The listing builds one solid part. Answer for the finished solid, in the listing's coordinates (mm). A direction names the side the tool comes from. Give positions to 0.01 mm unless a question says otherwise; leave off trailing zeros. Order: outer loops, then holes, each group sorted by start corner. A loop starts at its lowest first (then second) coordinate and runs counter-clockwise, first axis right, second up. Notation, with made-up numbers: (43, -11.75) -> (58, -11.75) arc R23 ccw to (58, 11.25) -> close; hole circle Ø6 at (-13.5, 48). An arc over 180 degrees is marked (long way). Write item = value, one per line. Start each with the question number.
```python
from build123d import *

# Parameters (mm, degrees)
SKETCH_1_W      = 130
SKETCH_1_H      = 130
SKETCH_1_R      = 5
EXTRUDE_1_DEPTH = 99
SKETCH_2_R      = 55
EXTRUDE_2_DEPTH = 5
SKETCH_3_R      = 11
EXTRUDE_3_DEPTH = 52
SKETCH_5_W      = 28.58431815
SKETCH_5_H      = 29.945476157
SKETCH_5_W_2    = 14.292159074
SKETCH_5_H_2    = 14.972738078
EXTRUDE_4_DEPTH = 86
SKETCH_6_R      = 40
EXTRUDE_5_DEPTH = 50


with BuildPart() as part:
    # 草图1 → 凸台-拉伸1 (new, symmetric)
    with BuildSketch(Plane.XY):
        Rectangle(SKETCH_1_W, SKETCH_1_H)
        with Locations((-51.265241636, 51.265241636)):
            Circle(SKETCH_1_R, mode=Mode.SUBTRACT)
        with Locations(Location((51.265241636, 51.265241636, 0), (0, 0, 180))):
            Circle(SKETCH_1_R, mode=Mode.SUBTRACT)
        with Locations(Location((-51.265241636, -51.265241636, 0), (0, 0, 180))):
            Circle(SKETCH_1_R, mode=Mode.SUBTRACT)
        with Locations((51.265241636, -51.265241636)):
            Circle(SKETCH_1_R, mode=Mode.SUBTRACT)
    extrude(amount=EXTRUDE_1_DEPTH, both=True)

    # 草图2 → 凸台-拉伸2 (add)
    with BuildSketch(Plane.XY.offset(99)):
        Circle(SKETCH_2_R)
    extrude(amount=EXTRUDE_2_DEPTH)

    # 草图3 → 凸台-拉伸3 (add)
    with BuildSketch(Plane.XY.offset(104)):
        with Locations(Location((0, 0, 0), (0, 0, 180))):
            Circle(SKETCH_3_R)
    extrude(amount=EXTRUDE_3_DEPTH)

    # 草图5 → 凸台-拉伸4 (add)
    with BuildSketch(Plane(origin=(0, 0, 0), x_dir=(1, 0, 0), z_dir=(0, 1, 0))):
        with Locations((0, 39.269782118)):
            Rectangle(SKETCH_5_W, SKETCH_5_H)
        with Locations((0, 82.486548844)):
            Rectangle(SKETCH_5_W_2, SKETCH_5_H_2)
    extrude(amount=EXTRUDE_4_DEPTH)

    # 草图6 → 凸台-拉伸5 (add)
    with BuildSketch(Plane(origin=(0, 0, -99), x_dir=(-1, 0, 0), z_dir=(0, 0, -1))):
        with Locations(Location((0, 0, 0), (0, 0, 180))):
            Circle(SKETCH_6_R)
    extrude(amount=EXTRUDE_5_DEPTH)


solid = part.part
```
Item 1: The mould has two halves that part along Z. Classify faces 1 (the flat face through (-59, 1, 99)), 2 (the flat face through (0, 75, -75)), 3 (the flat face through (-7.146, 75, -82)): +Z half, -Z half, draft (parallel to the pull), parting line (faces both ways), or undercut.
Item 2: Which of the six approach directions +Z, -Z, +X, -X, +Y, -Y give full straight-line access (tool end or side, diameter ignored) to faces 4 (the flat face through (-14.292, 75, -39)), 5 (the flat face through (14.292, 75, -39)), 6 (the cylindrical face through (2.38, 10.74, 129.64))?
Item 3: A cutting plane is placed at C-C, the plane x = 0. Write down the section's boundary in (y, z).
Item 4: A cutting plane is placed at A-A, the plane y = 75. Write down the section's boundary in (x, z), plus the area to 3 significant figures.
Item 5: Consider L1, parallel to Y at x = -0.5, z = -107; L2, parallel to Y at x = -19, z = 71.5; L3, parallel to Z at x = -9.5, y = 77. Determine where each line is inside the solid, lowest interval first. Write a range as from..to.
Item 6: A cutting plane is placed at B-B, the plane z = -79. Write down the section's boundary in (x, y).
Item 7: A cutting plane is placed at D-D, the plane y = 0. Write down the section's boundary in (x, z), plus the area to 3 significant figures.
Item 8: Flat-ended cylindrical pins translate along their axes: pin 1 (12 mm diameter, centred on x = 20.5, y = -5.5, fed in from +Z); pin 2 (10.5 mm diameter, centred on x = 3, y = 77, fed in from +Z); pin 3 (16 mm diameter, centred on x = 51.27, y = -51.27, fed in from +Z). Find the tip coordinate at first contact, or state that the pin passes through.
Check values:
q1.face_1 = +Z half
q1.face_2 = undercut
q1.face_3 = draft
q2.face_4 = +Z, -Z, -X, +Y
q2.face_5 = +Z, -Z, +X, +Y
q2.face_6 = +Z
q3.outline = (-65, -99) -> (-40, -99) -> (-40, -149) -> (40, -149) -> (40, -99) -> (65, -99) -> (65, -89.97) -> (86, -89.97) -> (86, -75) -> (65, -75) -> (65, -54.24) -> (86, -54.24) -> (86, -24.3) -> (65, -24.3) -> (65, 99) -> (55, 99) -> (55, 104) -> (11, 104) -> (11, 156) -> (-11, 156) -> (-11, 104) -> (-55, 104) -> (-55, 99) -> (-65, 99) -> close
q4.outline = (-14.29, -54.24) -> (14.29, -54.24) -> (14.29, -24.3) -> (-14.29, -24.3) -> close; (-7.15, -89.97) -> (7.15, -89.97) -> (7.15, -75) -> (-7.15, -75) -> close
q4.area = 1,070 mm^2
q5.L1 = -40..40
q5.L2 = -65..65
q5.L3 = -54.24..-24.3
q6.outline = (-65, -65) -> (65, -65) -> (65, 65) -> (7.15, 65) -> (7.15, 86) -> (-7.15, 86) -> (-7.15, 65) -> (-65, 65) -> close; hole circle Ø10 at (-51.27, -51.27); hole circle Ø10 at (-51.27, 51.27); hole circle Ø10 at (51.27, -51.27); hole circle Ø10 at (51.27, 51.27)
q7.outline = (-65, -99) -> (-40, -99) -> (-40, -149) -> (40, -149) -> (40, -99) -> (65, -99) -> (65, 99) -> (55, 99) -> (55, 104) -> (11, 104) -> (11, 156) -> (-11, 156) -> (-11, 104) -> (-55, 104) -> (-55, 99) -> (-65, 99) -> close
q7.area = 31,400 mm^2
q8.pin_1 = 104
q8.pin_2 = -24.3
q8.pin_3 = 99
